Input: part model. Units: mm. Frame: model coordinates. Give positions to 0.01 mm unless a question says otherwise; leave off trailing zeros. Loops run counter-clockwise (first coordinate to the right, second up) from the corner with the lowest first, then second, coordinate; pieces in that order, holes last. Notation, with made-up numbers: (71, -27.75) - (79, -27.75) arc R26 ccw to (79, -12.75) - close; hole circle Ø11 at (56.5, 0.5). An arc over 180 degrees is marked (long way). One line per item, written item: value.
from build123d import *

# Parameters (mm, degrees)
BOSS_EXTRUDE2_DEPTH = 3.5
SKETCH4_R           = 3.674588618
CUT_EXTRUDE1_DEPTH  = 10
SKETCH2_R           = 3.674588618
CUT_EXTRUDE2_DEPTH  = 10


with BuildPart() as part:
    # Sketch1 → Boss-Extrude2 (new, symmetric)
    with BuildSketch(Plane.XY):
        with BuildLine():
            Line((-32.510632707, 16.288746435), (-32.510632707, 0))
            ThreePointArc((-32.510632707, 0), (-27.065651732, -5.444980975), (-21.620670757, 0))
            Line((-21.620670757, 0), (-21.620670757, 16.288746435))
            ThreePointArc((-21.620670757, 16.288746435), (-27.065651732, 21.73372741), (-32.510632707, 16.288746435))
        make_face()
    extrude(amount=BOSS_EXTRUDE2_DEPTH, both=True)

    # Sketch4 → Cut-Extrude1 (cut)
    with BuildSketch(Plane.XY.offset(3.5)):
        with Locations((-27.065651732, 0)):
            Circle(SKETCH4_R)
    extrude(amount=-CUT_EXTRUDE1_DEPTH, mode=Mode.SUBTRACT)

    # Sketch2 → Cut-Extrude2 (cut)
    with BuildSketch(Plane.XY.offset(3.5)):
        with Locations((-27.065651732, 16.288746435)):
            Circle(SKETCH2_R)
    extrude(amount=-CUT_EXTRUDE2_DEPTH, mode=Mode.SUBTRACT)


solid = part.part
Item 1: Pin query (flat end, axial travel): P1, Ø6.5, axis at x = -27.07, y = 0, coming from the +Z side; P2, Ø1.5, axis at x = -26, z = -0.5, coming from the +Y side. Return the tip coordinate at first contact, or that it passes through.
Verdict:
P1: passes through
P2: stops at y = 21.72
Item 2: Section D-D, the plane x = -27.75. Output: boundary loops of the cut face in (y, z).
Verdict:
outline: (-5.4, -3.5) - (-3.61, -3.5) - (-3.61, 3.5) - (-5.4, 3.5) - close; (3.61, -3.5) - (12.68, -3.5) - (12.68, 3.5) - (3.61, 3.5) - close; (19.9, -3.5) - (21.69, -3.5) - (21.69, 3.5) - (19.9, 3.5) - close
Item 3: Draft query along Z for faces 1 (the face through (-21.621, 8, 0)), 2 (the face through (-27, 8, -3.5)), 3 (the face through (-27, 8, 3.5)). Return one class per face: pulls with the +Z half, pulls with the -Z half, needs draft (parallel to the pull), parting line crosses it, or undercut.
Verdict:
face 1: needs draft
face 2: pulls with the -Z half
face 3: pulls with the +Z half
Item 4: Section A-A, the plane y = -0.75. Output: boundary loops of the cut face in (x, z), and give its area (3 significant figures).
Verdict:
outline: (-32.46, -3.5) - (-30.66, -3.5) - (-30.66, 3.5) - (-32.46, 3.5) - close; (-23.47, -3.5) - (-21.67, -3.5) - (-21.67, 3.5) - (-23.47, 3.5) - close
area: 25.1 mm^2
Item 5: Section B-B, the plane x = -24.5. Output: boundary loops of the cut face in (y, z), and give its area (3 significant figures).
Verdict:
outline: (-4.8, -3.5) - (-2.63, -3.5) - (-2.63, 3.5) - (-4.8, 3.5) - close; (2.63, -3.5) - (13.66, -3.5) - (13.66, 3.5) - (2.63, 3.5) - close; (18.92, -3.5) - (21.09, -3.5) - (21.09, 3.5) - (18.92, 3.5) - close
area: 108 mm^2
Item 6: Material intervals for L1, parallel to Y at x = -30, z = -1.5; L2, parallel to Y at x = -24.75, z = -1.5; L3, parallel to X at y = 1.75, z = -1.75, sorted ascending.
Verdict:
L1: y = -4.59 to -2.21, 2.21 to 14.08, 18.5 to 20.88
L2: y = -4.93 to -2.85, 2.85 to 13.44, 19.14 to 21.22
L3: x = -32.51 to -30.3, -23.83 to -21.62
Item 7: Section C-C, the plane z = 0. Output: boundary loops of the cut face in (x, y), and give its area (3 significant figures).
Verdict:
outline: (-32.51, 0) arc R5.44 ccw to (-21.62, 0) - (-21.62, 16.29) arc R5.44 ccw to (-32.51, 16.29) - close; hole circle Ø7.35 at (-27.07, 0); hole circle Ø7.35 at (-27.07, 16.29)
area: 186 mm^2
